from build123d import *

# Parameters (mm, degrees)
EXTRUDE_1_DEPTH          = 20
SKETCH_2_W               = 30
SKETCH_2_H               = 37
CUT_EXTRUDE_1_DEPTH      = 20
CUT_EXTRUDE_2_DEPTH      = 157.04887055
CUT_EXTRUDE_2_DEPTH_BACK = 157.04887055
SKETCH_3_R               = 6
CUT_EXTRUDE_3_DEPTH      = 138.362886181
CUT_EXTRUDE_3_DEPTH_BACK = 138.362886181
SKETCH_4_W               = 85.5
SKETCH_4_H               = 10
SKETCH_5_W               = 85.5
SKETCH_5_H               = 20
CUT_EXTRUDE_4_DEPTH      = 8.43
EXTRUDE_START            = -20
SKETCH_6_W               = 85.5
SKETCH_6_H               = 4
EXTRUDE_2_DEPTH          = 90
SKETCH_8_R               = 3
CUT_EXTRUDE_6_DEPTH      = 90
FILLET_1_R               = 1
SKETCH_9_R               = 37.5
CUT_EXTRUDE_7_DEPTH      = 1.5
CUT_EXTRUDE_8_DEPTH      = 195.524927451
CUT_EXTRUDE_8_DEPTH_BACK = 195.524927451
SKETCH_10_R              = 7.75
SKETCH_11_R              = 10
CUT_EXTRUDE_9_DEPTH      = 1.5


with BuildPart() as part:
    # 草图1 → 凸台-拉伸1 (new body)
    with BuildSketch(Plane.XY):
        Polygon((-42.75, -59), (-42.75, 59), (-42.75, 129), (42.75, 129), (42.75, 59), (42.75, -59), align=None)
    extrude(amount=EXTRUDE_1_DEPTH)

    # 草图2 → 切除-拉伸1 (cut)
    with BuildSketch(Plane.XY.offset(20)):
        with Locations((-0.051962385, 110.5)):
            Rectangle(SKETCH_2_W, SKETCH_2_H)
    extrude(amount=-CUT_EXTRUDE_1_DEPTH, mode=Mode.SUBTRACT)

    # 草图3 → 切除-拉伸2 (cut, two sides: drawn at the far end of the back side and taken through both)
    with BuildSketch(Plane.ZY.offset(42.75).offset(-CUT_EXTRUDE_2_DEPTH_BACK)):
        with Locations((10, 114)):
            Circle(SKETCH_3_R)
    extrude(amount=CUT_EXTRUDE_2_DEPTH + CUT_EXTRUDE_2_DEPTH_BACK, mode=Mode.SUBTRACT)

    # 草图4 → 切除-拉伸3 (cut, two sides: drawn at the far end of the back side and taken through both)
    with BuildSketch(Plane.XY.offset(20).offset(-CUT_EXTRUDE_3_DEPTH_BACK)):
        with Locations((0, -54)):
            Rectangle(SKETCH_4_W, SKETCH_4_H)
    extrude(amount=CUT_EXTRUDE_3_DEPTH + CUT_EXTRUDE_3_DEPTH_BACK, mode=Mode.SUBTRACT)

    # 草图5 → 切除-拉伸4 (cut)
    with BuildSketch(Plane.XZ.offset(49)):
        with Locations((0, 10)):
            Rectangle(SKETCH_5_W, SKETCH_5_H)
    extrude(amount=-CUT_EXTRUDE_4_DEPTH, mode=Mode.SUBTRACT)

    # 草图6 → 凸台-拉伸2 (add)
    with BuildSketch(Plane.XY.offset(20).offset(EXTRUDE_START)):
        with Locations((0, -38.57)):
            Rectangle(SKETCH_6_W, SKETCH_6_H)
    extrude(amount=-EXTRUDE_2_DEPTH)

    # 草图8 → 切除-拉伸6 (cut)
    with BuildSketch(Plane(origin=(0, -36.57, 0), x_dir=(1, 0, 0), z_dir=(0, 1, 0))):
        with Locations(Location((-34.8, 77.55, 0), (0, 0, 270))):
            Circle(SKETCH_8_R)
        with Locations(Location((34.8, 77.55, 0), (0, 0, 270))):
            Circle(SKETCH_8_R)
        with Locations(Location((-34.8, 7.95, 0), (0, 0, 270))):
            Circle(SKETCH_8_R)
        with Locations(Location((34.8, 7.95, 0), (0, 0, 270))):
            Circle(SKETCH_8_R)
    extrude(amount=-CUT_EXTRUDE_6_DEPTH, mode=Mode.SUBTRACT)

    # 圆角1
    fillet_1_edges = [part.edges().sort_by_distance(p)[0] for p in [
        (0, -36.57, 0),
    ]]
    fillet(fillet_1_edges, radius=FILLET_1_R)

    # 草图9 → 切除-拉伸7 (cut)
    with BuildSketch(Plane(origin=(0, -36.57, 0), x_dir=(1, 0, 0), z_dir=(0, 1, 0))):
        with Locations(Location((0, 42.75, 0), (0, 0, 270))):
            Circle(SKETCH_9_R)
    extrude(amount=-CUT_EXTRUDE_7_DEPTH, mode=Mode.SUBTRACT)

    # 草图10 → 切除-拉伸8 (cut, two sides: drawn at the far end of the back side and taken through both)
    with BuildSketch(Plane(origin=(0, -38.07, 0), x_dir=(1, 0, 0), z_dir=(0, 1, 0)).offset(-CUT_EXTRUDE_8_DEPTH_BACK)):
        with Locations(Location((0, 42.75, 0), (0, 0, 270))):
            Circle(SKETCH_10_R)
    extrude(amount=CUT_EXTRUDE_8_DEPTH + CUT_EXTRUDE_8_DEPTH_BACK, mode=Mode.SUBTRACT)

    # 草图11 → 切除-拉伸9 (cut)
    with BuildSketch(Plane(origin=(0, -38.07, 0), x_dir=(1, 0, 0), z_dir=(0, 1, 0))):
        with Locations(Location((0, 42.75, 0), (0, 0, 270))):
            Circle(SKETCH_11_R)
    extrude(amount=-CUT_EXTRUDE_9_DEPTH, mode=Mode.SUBTRACT)


solid = part.part
Read the model definition and answer for the solid it produces. Units are mm, in the model's axes. A direction names the side the tool comes from. Give positions to 0.01 mm unless a question says otherwise; leave off trailing zeros. Write each loop counter-clockwise with the first axis right and the second up, starting at its lowest first coordinate (ties: lowest second). Pieces come first, ordered by that corner, then holes. Notation, with made-up numbers: M 34,20 L 47,20 A19 cw 47,51 Z; hole C 82,-37.5 d1. An arc over 180 degrees is marked long. One line per item, written item: value. Start each with the question number.
(1) Determine the mould class of faces 1 (the cylindrical face through (0.44, -38.81, -52.74)), 2 (the flat face through (-42.75, 31, 6)), 3 (the flat face through (-1, -39, -90)) for opening direction X: pulls with the +X half, pulls with the -X half, needs draft (parallel to the pull), parting line crosses it, or undercut.
(2) A tool of negligible diameter and unlimited length cuts with its end or side. For faces 4 (the flat face through (-39, -36.57, -45)), 5 (the flat face through (-15.052, 106, 10)), 6 (the cylindrical face through (11.26, -37.31, -6.98)), from which of +Z, -Z, +X, -X, +Y, -Y can it reach the whole face along a straight path? Write none if from no direction.
(3) Find the intervals of material crossed by line 1 (X direction, y = -39.2, z = -7.95); line 2 (Z direction, x = -27.5, y = 114); line 3 (Y direction, x = 24, z = 10), in increasing order.
(4) Flat-ended cylindrical pins translate along their axes: pin 1 Ø5 at (x, z) = (34.8, -7.95) entering from -Y; pin 2 Ø8 at (x, z) = (-8.5, -34) entering from +Y; pin 3 Ø1 at (x, y) = (6, 73) entering from -Z; pin 4 Ø10 at (x, z) = (-1, -46.5) entering from +Y. Find the tip coordinate at first contact, or state that the pin passes through.
(5) Find section B-B (x = -34.8). Determine the outline of the cut face in (y, z), plus the area to 3 significant figures.
(6) Find section A-A (z = -42.75). Determine the outline of the cut face in (x, y).
(7) Find section D-D (z = -7.95). Determine the outline of the cut face in (x, y), plus the area to 3 significant figures.
(8) Find section C-C (y = 102). Determine the outline of the cut face in (x, z).
Results below:
1. face 1: undercut
1. face 2: pulls with the -X half
1. face 3: needs draft
2. face 4: -Z, +X, -X, +Y
2. face 5: +Z, -Z, +Y
2. face 6: +Y
3. line 1: x = -42.75 to -37.8, -31.8 to 31.8, 37.8 to 42.75
3. line 2: z = 0 to 4, 16 to 20
3. line 3: y = -40.57 to 108, 120 to 129
4. pin 1: passes through
4. pin 2: stops at y = -38.07
4. pin 3: stops at z = 0
4. pin 4: stops at y = -39.57
5. outline: M -40.57,-90 L -36.57,-90 L -36.57,-80.55 L -40.57,-80.55 Z; M -40.57,-74.55 L -36.57,-74.55 L -36.57,-56.72 L -38.07,-56.72 L -38.07,-28.78 L -36.57,-28.78 L -36.57,-10.95 L -40.57,-10.95 Z; M -40.57,-4.95 L -36.57,-4.95 L -36.57,-1 A1 cw -35.57,0 L 129,0 L 129,20 L -40.57,20 Z; hole C 114,10 d12
5. area: 3,550 mm^2
6. outline: M -42.75,-40.57 L -7.75,-40.57 L -7.75,-39.57 L -10,-39.57 L -10,-38.07 L -37.5,-38.07 L -37.5,-36.57 L -42.75,-36.57 Z; M 7.75,-40.57 L 42.75,-40.57 L 42.75,-36.57 L 37.5,-36.57 L 37.5,-38.07 L 10,-38.07 L 10,-39.57 L 7.75,-39.57 Z
7. outline: M -42.75,-40.57 L -37.8,-40.57 L -37.8,-36.57 L -42.75,-36.57 Z; M -31.8,-40.57 L 31.8,-40.57 L 31.8,-36.57 L 13.97,-36.57 L 13.97,-38.07 L -13.97,-38.07 L -13.97,-36.57 L -31.8,-36.57 Z; M 37.8,-40.57 L 42.75,-40.57 L 42.75,-36.57 L 37.8,-36.57 Z
7. area: 252 mm^2
8. outline: M -42.75,0 L -15.05,0 L -15.05,20 L -42.75,20 Z; M 14.95,0 L 42.75,0 L 42.75,20 L 14.95,20 Z
